Study the drawing (mm; zero at the part's minimum x, y, z) and answer. A direction names the side the tool comes from. Coordinates: 2 decimals unless noted, no trailing zeros. Write each loop counter-clockwise with the first axis right and the second up, starting at its lowest first coordinate (ties: lowest second). Pieces come first, ordered by that corner, then holes. Notation, with made-up numbers: M 43,73 L 49,73 A31 cw 49,106 Z; hole C 60.25,5.5 d6. An arc over 180 degrees is marked long. Answer as CSV lines item,"result". Start each with the question number.
(1) Flat-ended cylindrical pins translate along their axes: P1, Ø8, axis at x = 21, y = 37, coming from the +Z side; P2, Ø1.5, axis at y = 16.5, z = 16, coming from the -X side; P3, Ø2, axis at x = 39.5, z = 44.5, coming from the -Y side. Find the tip coordinate at first contact, or state that the pin passes through.
(2) A cutting plane is placed at C-C on y = 40.5. Give the vertices of the cut face in (x, z), then the cut area to 3 significant figures.
(3) A cutting plane is placed at A-A on z = 25. Give the vertices of the cut face in (x, y).
(4) For the marked faces 4 and 5, determine the directions among +Z, -Z, +X, -X, +Y, -Y from which every point of the face is accessible in a straight line to the end or side of a thin tool.
(5) The mould has two halves that part along Y. Classify the marked faces 1, 2 and 3: released by +Y, released by -Y, zero draft, split by the parting line, or undercut.
(6) A cutting plane is placed at D-D on y = 22. Give the vertices of the cut face in (x, z), then the cut area to 3 significant figures.
(7) A cutting plane is placed at B-B on x = 25. Give the vertices of the cut face in (y, z).
(8) Find the intervals of material crossed by L1, parallel to Y at x = 30, z = 42; L2, parallel to Y at x = 11, z = 41; L3, parallel to X at y = 22, z = 30.5, in increasing order. Write a range as [from, to].
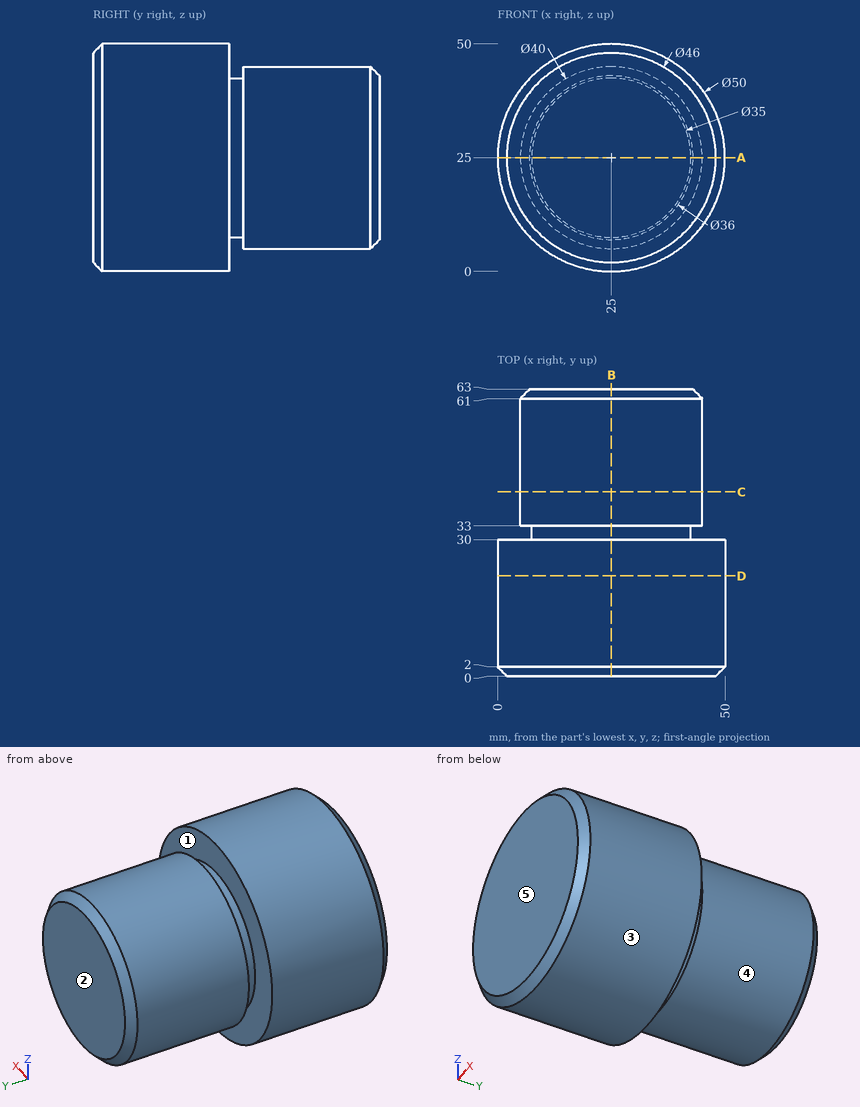
Here are the results:
1,P1,"stops at z = 45"
1,P2,"stops at x = 1.4"
1,P3,"stops at y = 0.3"
2,outline,"C 25,25 d40"
2,area,"1,260 mm^2"
3,outline,"M 0,2 L 2,0 L 48,0 L 50,2 L 50,30 L 42.5,30 L 42.5,33 L 45,33 L 45,61 L 43,63 L 7,63 L 5,61 L 5,33 L 7.5,33 L 7.5,30 L 0,30 Z"
4,face 4,"+Y"
4,face 5,"+Z, -Z, +X, -X, -Y"
5,face 1,"undercut"
5,face 2,"released by +Y"
5,face 3,"zero draft"
6,outline,"C 25,25 d50"
6,area,"1,960 mm^2"
7,outline,"M 0,2 L 2,0 L 30,0 L 30,7.5 L 33,7.5 L 33,5 L 61,5 L 63,7 L 63,43 L 61,45 L 33,45 L 33,42.5 L 30,42.5 L 30,50 L 2,50 L 0,48 Z"
8,L1,"y = [0, 30], [33, 63]"
8,L2,"y = [0, 30]"
8,L3,"x = [0.61, 49.39]"
